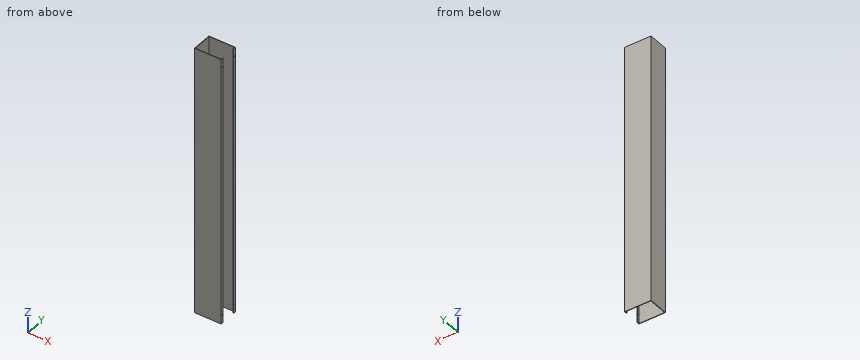
from build123d import *

# Parameters (mm, degrees)
EXTRUDE_1_DEPTH         = 800
HOLE_WIZARD_M3_1_REACH  = 808.078
HOLE_WIZARD_M3_1_BORE_R = 1.25


with BuildPart() as part:
    # Sketch 1 → Extrude 1 (new body)
    with BuildSketch(Plane.XY):
        Polygon((78.5, 52), (78.5, 60), (0, 60), (0, 0), (78.5, 0), (78.5, 8), (77, 8), (77, 1.5), (1.5, 1.5), (1.5, 58.5), (77, 58.5), (77, 52), align=None)
    extrude(amount=EXTRUDE_1_DEPTH)

    # Hole Wizard M3 _1 bore → Hole Wizard M3 _1 (cut, up to next)
    with BuildSketch(Plane(origin=(78.5, 0, 0), x_dir=(0, 0, -1), z_dir=(1, 0, 0)), mode=Mode.PRIVATE) as hole_wizard_m3_1_sk1:
        with Locations((-775, 56)):
            Circle(HOLE_WIZARD_M3_1_BORE_R)
    hole_wizard_m3_1_tool1 = extrude(hole_wizard_m3_1_sk1.sketch, amount=-HOLE_WIZARD_M3_1_REACH, mode=Mode.PRIVATE) & part.part
    # Hole Wizard M3 _1 bore → Hole Wizard M3 _1 (cut, up to next)
    with BuildSketch(Plane(origin=(78.5, 0, 0), x_dir=(0, 0, -1), z_dir=(1, 0, 0)), mode=Mode.PRIVATE) as hole_wizard_m3_1_sk2:
        with Locations((-25, 56)):
            Circle(HOLE_WIZARD_M3_1_BORE_R)
    hole_wizard_m3_1_tool2 = extrude(hole_wizard_m3_1_sk2.sketch, amount=-HOLE_WIZARD_M3_1_REACH, mode=Mode.PRIVATE) & part.part
    hole_wizard_m3_1_1 = hole_wizard_m3_1_tool1.solids().sort_by_distance((78.5, 56, 775))[0]
    add(hole_wizard_m3_1_1, mode=Mode.SUBTRACT)
    hole_wizard_m3_1_2 = hole_wizard_m3_1_tool2.solids().sort_by_distance((78.5, 56, 25))[0]
    add(hole_wizard_m3_1_2, mode=Mode.SUBTRACT)
    hole_wizard_m3_1 = hole_wizard_m3_1_1 + hole_wizard_m3_1_2  # Hole Wizard M3 _1 as one shape, for the pattern or mirror that repeats it

    # Mirror 2: Hole Wizard M3 _1 across plane
    add(hole_wizard_m3_1.mirror(Plane(origin=(0, 30, 0), x_dir=(0, 0, 1), z_dir=(0, -1, 0))), mode=Mode.SUBTRACT)


solid = part.part
Could you check a few things on this model? Use its own coordinates, in mm. Give positions to 0.01 mm unless a question says otherwise; leave off trailing zeros. Order: outer loops, then holes, each group sorted by start corner. A loop starts at its lowest first (then second) coordinate and runs counter-clockwise, first axis right, second up.
1. Will this pin go through, and if not, where does the flat tip stop? P1, Ø2, axis at y = 4, z = 25, coming from the +X side.
2. Suppose I cut it at A-A (x = 47). List the corners of the cut face in (y, z) for me, plus the area to 3 significant figures.
3. I need wall thicknesses on L1, parallel to Y at x = 77.8, z = 775; L2, parallel to Z at x = 77.65, y = 4; L3, parallel to Y at x = 44, z = 180. Which ranges of each line are inside material? Lowest first, please.
4. Suppose I cut it at B-B (z = 215.5). List the corners of the cut face in (x, y) for me, plus the area to 4 significant figures.
5. Suppose I cut it at C-C (y = 44). List the corners of the cut face in (x, z) for me.
Solved:
1. P1: stops at x = 1.5
2. outline: (0, 0) - (1.5, 0) - (1.5, 800) - (0, 800) - close; (58.5, 0) - (60, 0) - (60, 800) - (58.5, 800) - close
2. area: 2,400 mm2
3. L1: y = 0 to 2.75, 5.25 to 8, 52 to 54.75, 57.25 to 60
3. L2: z = 0 to 23.75, 26.25 to 773.75, 776.25 to 800
3. L3: y = 0 to 1.5, 58.5 to 60
4. outline: (0, 0) - (78.5, 0) - (78.5, 8) - (77, 8) - (77, 1.5) - (1.5, 1.5) - (1.5, 58.5) - (77, 58.5) - (77, 52) - (78.5, 52) - (78.5, 60) - (0, 60) - close
4. area: 340.5 mm2
5. outline: (0, 0) - (1.5, 0) - (1.5, 800) - (0, 800) - close
